from build123d import *

# Parameters (mm, degrees)
GB_T_707_1988_HOT_ROLLED_CHANNEL_05_1_DEPTH = 1000
CUT_EXTRUDE6_DEPTH                          = 504.854145562
CUT_EXTRUDE6_DEPTH_BACK                     = 504.854145562


with BuildPart() as part:
    # Sketch1 → GB/T 707-1988 hot-rolled channel 05(1) (new body)
    with BuildSketch(Plane.YZ.offset(-500)):
        with BuildLine():
            Line((37, 50), (0, 50))
            Line((0, 50), (0, 0))
            Line((0, 0), (37, 0))
            Line((37, 0), (37, 2.140642022))
            ThreePointArc((37, 2.140642022), (36.101006889, 4.482599144), (33.865849621, 5.621468656))
            Line((33.865849621, 5.621468656), (10.768300757, 8.049118866))
            ThreePointArc((10.768300757, 8.049118866), (6.297986222, 10.326857889), (4.5, 15.010772133))
            Line((4.5, 15.010772133), (4.5, 34.989227867))
            ThreePointArc((4.5, 34.989227867), (6.297986222, 39.673142111), (10.768300757, 41.950881134))
            Line((10.768300757, 41.950881134), (33.865849621, 44.378531344))
            ThreePointArc((33.865849621, 44.378531344), (36.101006889, 45.517400856), (37, 47.859357978))
            Line((37, 47.859357978), (37, 50))
        make_face()
    extrude(amount=GB_T_707_1988_HOT_ROLLED_CHANNEL_05_1_DEPTH)

    # Sketch4 → Cut-Extrude6 (cut, two sides: drawn at the far end of the back side and taken through both)
    with BuildSketch(Plane.XZ.offset(-CUT_EXTRUDE6_DEPTH_BACK)):
        Polygon((-500, 50), (-500, 0), (-492.972958265, 50), align=None)
        Polygon((500, 50), (-34.511240341, 50), (-41.538282077, 0), (500, 0), align=None)
    extrude(amount=CUT_EXTRUDE6_DEPTH + CUT_EXTRUDE6_DEPTH_BACK, mode=Mode.SUBTRACT)


solid = part.part
Can you work these out from the model? Positions are in its coordinate system, mm. A direction names the side the tool comes from. Coordinates: 2 decimals unless noted, no trailing zeros. Order: outer loops, then holes, each group sorted by start corner. A loop starts at its lowest first (then second) coordinate and runs counter-clockwise, first axis right, second up. Notation, with made-up numbers: (75.25, -15) - (131.25, -15) arc R19 cw to (131.25, -5) - close; hole circle Ø11 at (56.25, 1.5). An arc over 180 degrees is marked (long way). Answer as a JSON object with one key per item and string values. Group by question number.
Q1. Imagine slicing it at B-B (x = -286). Please give me the cut outline in (y, z).
Q2. Will these pins go through, and if not, where does the flat tip stop? P1, Ø2, axis at x = -421, y = 14.5, coming from the -Z side; P2, Ø6, axis at x = -260, z = 20, coming from the +Y side.
Q3. Imagine slicing it at A-A (y = 27). Please give me the cut outline in (x, z).
Q4. On a 3-axis mill with a long thin cutter (end or side, diameter ignored), from which of +Z, -Z, +X, -X, +Y, -Y can I reach the whole of each face in a straight line? I mean faces 4 (the face through (-267.91, 22.16, 43.15)), 5 (the face through (-496.5, 3.5, 24.9)). Say none if no direction works.
Q5. We'd pull the mould along Z, two halves only. Please class faces 1 (the face through (-273.02, 22.48, 6.82)), 2 (the face through (-271, 0, 25)), 3 (the face through (-38.008, 3.512, 25.117)): +Z half, -Z half, draft (parallel to the pull), parting line (faces both ways), or undercut.
Q6. I need wall thicknesses on line 1 (Y direction, x = -121, z = 15); line 2 (X direction, y = 3.5, z = 14.5); line 3 (Z direction, x = -84.5, y = 7). Which ranges of each line are inside material? Lowest first, please. Write a range as from..to.
Q7. Imagine slicing it at C-C (z = 19). Please give me the cut outline in (x, y), and give its area (3 significant figures).
Determined:
{
 "1": {"outline": "(0, 0) - (37, 0) - (37, 2.14) arc R3.5 ccw to (33.87, 5.62) - (10.77, 8.05) arc R7 cw to (4.5, 15.01) - (4.5, 34.99) arc R7 cw to (10.77, 41.95) - (33.87, 44.38) arc R3.5 ccw to (37, 47.86) - (37, 50) - (0, 50) - close"},
 "2": {"P1": "stops at z = 0", "P2": "stops at y = 4.5"},
 "3": {"outline": "(-500, 0) - (-41.54, 0) - (-40.65, 6.34) - (-499.11, 6.34) - close; (-493.86, 43.66) - (-35.4, 43.66) - (-34.51, 50) - (-492.97, 50) - close"},
 "4": {"face 4": "+X, -X, +Y", "face 5": "+Z, -X, +Y, -Y"},
 "5": {"face 1": "undercut", "face 2": "draft", "face 3": "-Z half"},
 "6": {"line 1": "y = 0..4.5", "line 2": "x = -497.96..-39.5", "line 3": "z = 0..9.65, 40.35..50"},
 "7": {"outline": "(-497.33, 0) - (-38.87, 0) - (-38.87, 4.5) - (-497.33, 4.5) - close", "area": "2,060 mm2"}
}
